from build123d import *

# Parameters (mm, degrees)
SKETCH1_W                    = 55
SKETCH1_H                    = 47
BOSS_EXTRUDE1_DEPTH          = 10
SKETCH4_W                    = 10
SKETCH4_H                    = 47
BOSS_EXTRUDE2_DEPTH          = 74
M8_CLEARANCE_HOLE1_D         = 9
M8_CLEARANCE_HOLE1_DEPTH     = 121
M8_CLEARANCE_HOLE1_TIP       = 2.703872786
CHAMFER1_SIZE                = 2
SKETCH8_R                    = 11.5
CUT_EXTRUDE1_DEPTH           = 30
CHAMFER2_SIZE                = 2
SIZE_MM_BLIND_DOWEL_HOLE_1_D = 6
CIRPATTERN1_COUNT            = 4


with BuildPart() as part:
    # Sketch1 → Boss-Extrude1 (new body)
    with BuildSketch(Plane.XY):
        Rectangle(SKETCH1_W, SKETCH1_H)
    extrude(amount=BOSS_EXTRUDE1_DEPTH)

    # Sketch4 → Boss-Extrude2 (add)
    with BuildSketch(Plane(origin=(0, 0, 0), x_dir=(-1, 0, 0), z_dir=(0, 0, -1))):
        with Locations((-22.5, 0)):
            Rectangle(SKETCH4_W, SKETCH4_H)
    extrude(amount=BOSS_EXTRUDE2_DEPTH)

    # M8 Clearance Hole1
    with Locations(Plane(origin=(0, 0, 0), x_dir=(-1, 0, 0), z_dir=(0, 0, -1))):
        with Locations((17.5, -15), (17.5, 15), (-9.5, -15), (-9.5, 15)):
            Hole(M8_CLEARANCE_HOLE1_D / 2, depth=M8_CLEARANCE_HOLE1_DEPTH)
            with Locations((0, 0, -(M8_CLEARANCE_HOLE1_DEPTH + M8_CLEARANCE_HOLE1_TIP / 2))):  # 118° drill point
                Cone(0, M8_CLEARANCE_HOLE1_D / 2, M8_CLEARANCE_HOLE1_TIP, mode=Mode.SUBTRACT)

    # Chamfer1
    chamfer1_edges = [part.edges().sort_by_distance(p)[0] for p in [
        (-27.5, -23.5, 5),
        (-27.5, 23.5, 5),
    ]]
    chamfer(chamfer1_edges, length=CHAMFER1_SIZE)

    # Sketch8 → Cut-Extrude1 (cut)
    with BuildSketch(Plane.ZY.offset(-17.5)):
        with Locations(Location((-50, 0, 0), (0, 0, 270))):
            Circle(SKETCH8_R)
    extrude(amount=-CUT_EXTRUDE1_DEPTH, mode=Mode.SUBTRACT)

    # Chamfer2
    chamfer2_edges = [part.edges().sort_by_distance(p)[0] for p in [
        (22.5, 23.5, -74),
        (22.5, -23.5, -74),
    ]]
    chamfer(chamfer2_edges, length=CHAMFER2_SIZE)

    # Size mm blind dowel hole 1 (through all)
    with Locations(Plane(origin=(0, 0, 0), x_dir=(-1, 0, 0), z_dir=(0, 0, -1))):
        with Locations((4, -15), (4, 15)):
            Hole(SIZE_MM_BLIND_DOWEL_HOLE_1_D / 2)

    # Sketch14 → Hole size (per socket head cap screw type)1 (revolve, cut)
    with BuildSketch(Plane(origin=(17.5, -17, -67), x_dir=(0, 0, 1), z_dir=(0, 1, 0))):
        Polygon((0, 0), (0, 34.732840043), (3.3, 32.75), (3.3, 5), (5.5, 5), (5.5, 0), align=None)
    hole_size_per_socket_head_cap_screw_typ = revolve(axis=Axis((11.15, -17, -67), (1, 0, 0)), mode=Mode.SUBTRACT)

    # CirPattern1: Hole size (per socket head cap screw type)1 ×4 about axis
    cirpattern1_axis = Axis((0, 0, -50), (1, 0, 0))
    for i in range(1, CIRPATTERN1_COUNT):
        add(hole_size_per_socket_head_cap_screw_typ.rotate(cirpattern1_axis, i * 360 / CIRPATTERN1_COUNT), mode=Mode.SUBTRACT)


solid = part.part
The listing builds one solid part. Answer for the finished solid, in the listing's coordinates (mm). A direction names the side the tool comes from. Coordinates: 2 decimals unless noted, no trailing zeros. Loops run counter-clockwise (first coordinate to the right, second up) from the corner with the lowest first, then second, coordinate; pieces in that order, holes last.
1) Determine the mould class of faces 4 (the face through (22.6, -22.5, -73)), 5 (the face through (24.96, 17.43, -70.27)), 6 (the face through (-27.5, 0, 5)) for opening direction Y: pulls with the +Y half, pulls with the -Y half, needs draft (parallel to the pull), parting line crosses it, or undercut.
2) Find section C-C on z = -33. Write down the section's boundary in (x, y).
3) Find section D-D on y = -17. Give the number of separate pieces and of enclosed holes in the cut face, then the cut area to 3 significant figures.
4) Flat-ended cylindrical pins translate along their axes: pin 1 Ø3.5 at (y, z) = (16.5, -33.5) entering from -X; pin 2 Ø11.5 at (x, y) = (-17.5, -15) entering from -Z; pin 3 Ø8 at (y, z) = (-16.5, -22.5) entering from -X; pin 4 Ø10.5 at (y, z) = (17, -67) entering from -X. Find the tip coordinate at first contact, or state that the pin passes through.
5) Find section A-A on x = -4. Write down the section's boundary in (y, z).
6) A tool of negligible diameter and unlimited length cuts with its end or side. For faces 1 (the face through (-20.82, 18.04, 5.07)), 2 (the face through (22.5, 17, -29)), 3 (the face through (17.5, 0, -28)), from which of +Z, -Z, +X, -X, +Y, -Y can it reach the whole face along a straight path? Write none if from no direction.
7) Find the intervals of material crossed by L1, parallel to Y at x = 20, z = -67; L2, parallel to Y at x = -17.5, z = 5.75; L3, parallel to Z at x = 25, y = -17, in increasing order.
8) Find section B-B on y = 0. Write down the section's boundary in (x, z), then the cut area to 3 significant figures.
Values:
1. face 4: pulls with the -Y half
1. face 5: undercut
1. face 6: needs draft
2. outline: (17.5, -23.5) - (27.5, -23.5) - (27.5, -20.3) - (22.5, -20.3) - (22.5, -22.5) - (17.5, -22.5) - close; (17.5, -11.5) - (22.5, -11.5) - (22.5, -13.7) - (27.5, -13.7) - (27.5, 13.7) - (22.5, 13.7) - (22.5, 11.5) - (17.5, 11.5) - close; (17.5, 22.5) - (22.5, 22.5) - (22.5, 20.3) - (27.5, 20.3) - (27.5, 23.5) - (17.5, 23.5) - close
3. separate pieces: 6
3. enclosed holes: 0
3. area: 908 mm2
4. pin 1: passes through
4. pin 2: stops at z = 0
4. pin 3: stops at x = 17.5
4. pin 4: stops at x = 22.5
5. outline: (-23.5, 0) - (-18, 0) - (-18, 10) - (-23.5, 10) - close; (-12, 0) - (12, 0) - (12, 10) - (-12, 10) - close; (18, 0) - (23.5, 0) - (23.5, 10) - (18, 10) - close
6. face 1: +Z, -Z
6. face 2: -X
6. face 3: -Z, -X, +Y, -Y
7. L1: y = -23.5 to -22.5, -11.5 to 11.5, 22.5 to 23.5
7. L2: y = -23.5 to -19.5, -10.5 to 10.5, 19.5 to 23.5
7. L3: z = -74 to -70.3, -63.7 to -36.3, -29.7 to 10
8. outline: (-27.5, 0) - (17.5, 0) - (17.5, -38.5) - (27.5, -38.5) - (27.5, 10) - (-27.5, 10) - close; (17.5, -74) - (27.5, -74) - (27.5, -61.5) - (17.5, -61.5) - close
8. area: 1,060 mm2
